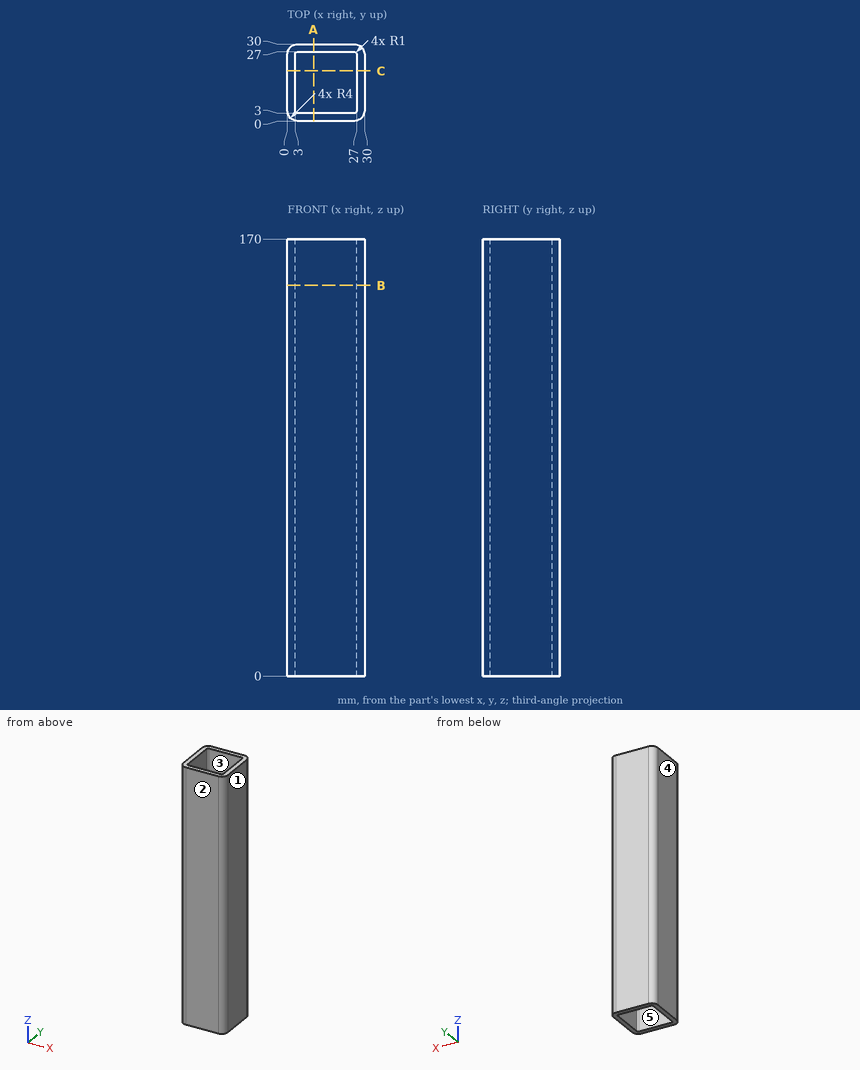
Design review of the part shown in the three views and the two pictorial views. Dimensions are in mm from the part's minimum x, y and z. A direction names the side the tool comes from. Round coordinates to 2 decimals unless told otherwise and drop trailing zeros. Order: outer loops, then holes, each group sorted by start corner. A loop starts at its lowest first (then second) coordinate and runs counter-clockwise, first axis right, second up. Notation, with made-up numbers: (33, 62.5) - (78, 62.5) arc R26 ccw to (78, 101.5) - close; hole circle Ø7 at (57.25, 74). An arc over 180 degrees is marked (long way). One line per question, with ' | ' between items.
Item 1: Take a section at B-B, the plane z = 152. Write out the cut boundary in (x, y).
Checks:
outline: (0, 4) arc R4 ccw to (4, 0) - (26, 0) arc R4 ccw to (30, 4) - (30, 26) arc R4 ccw to (26, 30) - (4, 30) arc R4 ccw to (0, 26) - close; hole (3, 4) arc R1 ccw to (4, 3) - (26, 3) arc R1 ccw to (27, 4) - (27, 26) arc R1 ccw to (26, 27) - (4, 27) arc R1 ccw to (3, 26) - close
Item 2: Take a section at A-A, the plane x = 10.25. Write out the cut boundary in (y, z), then the cut area to 3 significant figures.
Checks:
outline: (0, 0) - (3, 0) - (3, 170) - (0, 170) - close; (27, 0) - (30, 0) - (30, 170) - (27, 170) - close | area: 1,020 mm²
Item 3: Machinability: for the marked faces 4 and 5, which of the approach directions +Z, -Z, +X, -X, +Y, -Y give a long, thin tool a straight path to every point of the face, cutting with its end or side? Answer none if there is none.
Checks:
face 4: +Z, -Z, -X, +Y, -Y | face 5: +Z, -Z
Item 4: For P1, Ø12, axis at x = 15.5, y = 9.5, coming from the +Z side, flat-tipped, find the tip position at first contact; note if it passes through.
Checks:
P1: through
Item 5: Draft analysis for pull direction Y (two halves, no side actions). For the marked faces 1, 2 and 3, state which applies: +Y half, -Y half, draft (parallel to the pull), parting line (faces both ways), or undercut.
Checks:
face 1: draft | face 2: -Y half | face 3: undercut
Item 6: Wall thickness on line 1 (Y direction, x = 24, z = 22.5); line 2 (Y direction, x = 2, z = 97.5): over which ranges is each line inside the solid? List them lowest first. Write a range as [from, to].
Checks:
line 1: [0, 3], [27, 30] | line 2: [0.54, 29.46]
